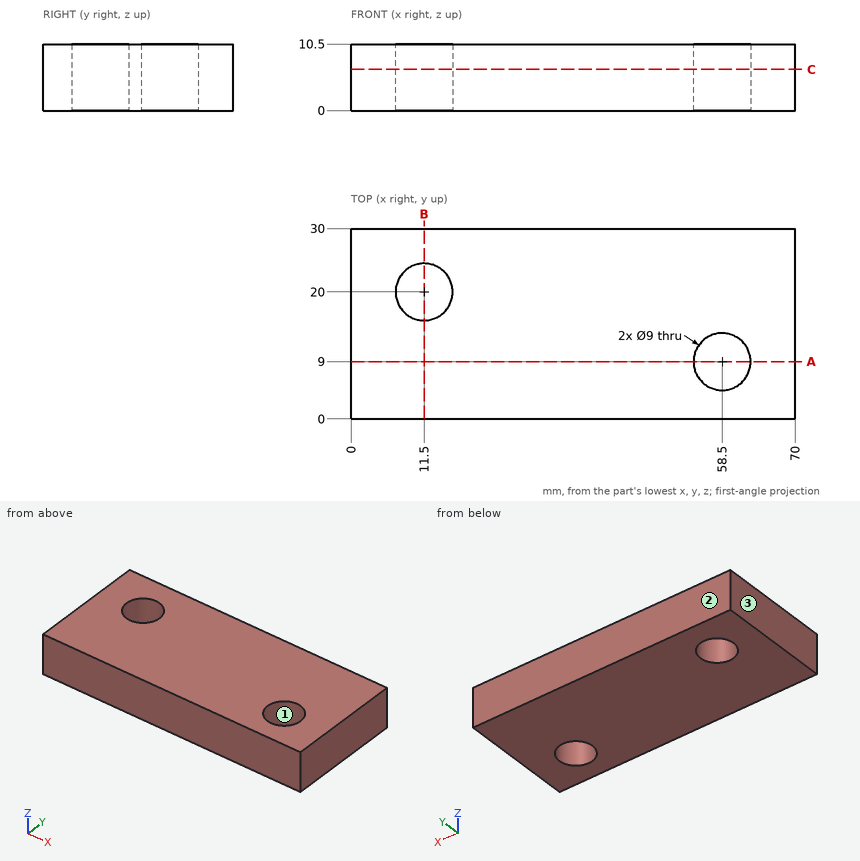
Geometry check sheet. Reference: drawing and pictorial views, mm from the part's lowest x, y, z. Round coordinates to 2 decimals unless told otherwise and drop trailing zeros. Order: outer loops, then holes, each group sorted by start corner. A loop starts at its lowest first (then second) coordinate and runs counter-clockwise, first axis right, second up.
Q1. Depth check by flat-ended pin: P1, Ø12, axis at x = 53, y = 16, coming from the -Z side. Enter the tip coordinate at first touch or a pass-through.
Filled sheet:
P1: stops at z = 0
Q2. Cross-section at B-B, the plane x = 11.5. Enter the section's corners in (y, z), plus the area to 4 significant figures.
Filled sheet:
outline: (0, 0) - (15.5, 0) - (15.5, 10.5) - (0, 10.5) - close; (24.5, 0) - (30, 0) - (30, 10.5) - (24.5, 10.5) - close
area: 220.5 mm2
Q3. Cross-section at A-A, the plane y = 9. Enter the section's corners in (x, z), plus the area to 4 significant figures.
Filled sheet:
outline: (0, 0) - (54, 0) - (54, 10.5) - (0, 10.5) - close; (63, 0) - (70, 0) - (70, 10.5) - (63, 10.5) - close
area: 640.5 mm2
Q4. Draft check along Y on the marked faces 1, 2 and 3. Enter one of: pulls with the +Y half, pulls with the -Y half, needs draft (parallel to the pull), parting line crosses it, or undercut.
Filled sheet:
face 1: undercut
face 2: pulls with the +Y half
face 3: needs draft
Q5. Scan lines: L1, parallel to Y at x = 11.5, z = 8.5; L2, parallel to X at y = 8.25, z = 8.25; L3, parallel to X at y = 9, z = 7.75. Record each from-to range of solid material in increasing order.
Filled sheet:
L1: y = 0 to 15.5, 24.5 to 30
L2: x = 0 to 54.06, 62.94 to 70
L3: x = 0 to 54, 63 to 70
Q6. Cross-section at C-C, the plane z = 6.5. Enter the section's corners in (x, y).
Filled sheet:
outline: (0, 0) - (70, 0) - (70, 30) - (0, 30) - close; hole circle Ø9 at (11.5, 20); hole circle Ø9 at (58.5, 9)
